```python
from build123d import *

# Parameters (mm, degrees)
SKETCH_1_R          = 13.5
EXTRUDE_1_DEPTH     = 60
SKETCH_4_R          = 13.05
EXTRUDE_3_DEPTH     = 17
CUT_EXTRUDE_2_REACH = 157.179
SKETCH_5_R          = 9
CHAMFER_1_SIZE      = 1


with BuildPart() as part:
    # 草图1 → 凸台-拉伸1 (new, symmetric)
    with BuildSketch(Plane.XY):
        Circle(SKETCH_1_R)
    extrude(amount=EXTRUDE_1_DEPTH, both=True)

    # 草图4 → 凸台-拉伸3 (add)
    with BuildSketch(Plane(origin=(0, 0, -60), x_dir=(-1, 0, 0), z_dir=(0, 0, -1))):
        Circle(SKETCH_4_R)
    extrude_3 = extrude(amount=EXTRUDE_3_DEPTH)

    # 镜向1: 凸台-拉伸3 across plane
    add(extrude_3.mirror(Plane.XY))

    # 草图5 → 切除-拉伸2 (cut, up to next)
    with BuildSketch(Plane(origin=(0, 0, -77), x_dir=(-1, 0, 0), z_dir=(0, 0, -1)), mode=Mode.PRIVATE) as cut_extrude_2_sk1:
        Circle(SKETCH_5_R)
    cut_extrude_2_tool1 = extrude(cut_extrude_2_sk1.sketch, amount=-CUT_EXTRUDE_2_REACH, mode=Mode.PRIVATE) & part.part
    add(cut_extrude_2_tool1.solids().sort_by_distance((0, 0, -77))[0], mode=Mode.SUBTRACT)

    # 倒角1
    chamfer_1_edges = [part.edges().sort_by_distance(p)[0] for p in [
        (13.05, 0, 77),
        (13.05, 0, -77),
    ]]
    chamfer(chamfer_1_edges, length=CHAMFER_1_SIZE)


solid = part.part
```
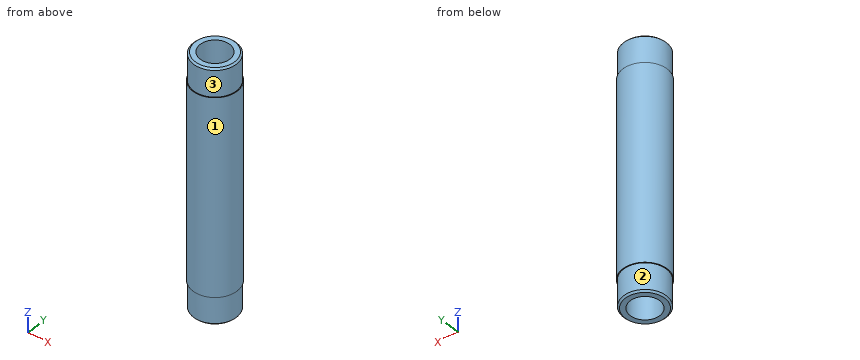
Geometry: final body of the model. Coordinates: model frame, mm. Face numbers are marked on the shaded views. A direction names the side the tool comes from. Coordinates: 2 decimals unless noted, no trailing zeros. Order: outer loops, then holes, each group sorted by start corner. A loop starts at its lowest first (then second) coordinate and runs counter-clockwise, first axis right, second up. Notation, with made-up numbers: (-30, 34.25) -> (9, 34.25) arc R15 ccw to (9, 58.25) -> close; hole circle Ø6 at (80, -31). An arc over 180 degrees is marked (long way). Write each question's results on one line, items separated by ' | '. Start each with the question number.
1) Cut plane A-A, the plane y = 0. Output: boundary loops of the cut face in (x, z).
2) Set-up query: the marked faces 1, 2 and 3. Return all of +Z, -Z, +X, -X, +Y, -Y with unobstructed straight access to the full face (end or side cutting, diameter ignored); none if empty.
3) Cut plane C-C, the plane z = -64.5. Output: boundary loops of the cut face in (x, y), and give its area (3 significant figures).
4) First-contact query: pin 1 (3 mm diameter, centred on x = 4, z = 3, fed in from +Y); pin 2 (5 mm diameter, centred on x = 8.5, z = -10, fed in from +Y); pin 3 (5 mm diameter, centred on y = -10, z = 36, fed in from +X) (3 decimals). Flat tips, straight axial feed; report the tip coordinate or a pass-through.
5) Cut plane D-D, the plane z = 54. Output: boundary loops of the cut face in (x, y).
6) Material intervals for line 1 along Y through (x, z) = (0, 23.5); line 2 along Y through (x, z) = (0, -67); line 3 along X through (y, z) = (-1.5, -42), sorted ascending.
Checks:
1) outline: (-13.5, -60) -> (-13.05, -60) -> (-13.05, -76) -> (-12.05, -77) -> (-9, -77) -> (-9, 77) -> (-12.05, 77) -> (-13.05, 76) -> (-13.05, 60) -> (-13.5, 60) -> close; (9, -77) -> (12.05, -77) -> (13.05, -76) -> (13.05, -60) -> (13.5, -60) -> (13.5, 60) -> (13.05, 60) -> (13.05, 76) -> (12.05, 77) -> (9, 77) -> close
2) face 1: +Z, -Z | face 2: -Z | face 3: +Z
3) outline: circle Ø26.1 at (0, 0); hole circle Ø18 at (0, 0) | area: 281 mm^2
4) pin 1: y = 13.27 | pin 2: y = 12.09 | pin 3: x = 11.225
5) outline: circle Ø27 at (0, 0); hole circle Ø18 at (0, 0)
6) line 1: -13.5 to -9, 9 to 13.5 | line 2: -13.05 to -9, 9 to 13.05 | line 3: -13.42 to -8.87, 8.87 to 13.42
